For this review, take the finished solid that the model builds, in its own axes (mm). A direction names the side the tool comes from. Round coordinates to 2 decimals unless told otherwise and drop trailing zeros.
from build123d import *

# Parameters (mm, degrees)
FILLET1_R = 40
FILLET2_R = 38
FILLET3_R = 16
FILLET4_R = 4


with BuildPart() as part:
    # Sketch1 → Revolve1 (revolve)
    with BuildSketch(Plane.XY, mode=Mode.PRIVATE) as revolve1_sk:
        Polygon((-150, 1.447982474), (-150, 24.174941718), (-52.599310337, 68.447982474), (0, 68.447982474), (0, 56.447982474), (-50, 56.447982474), (-132, 19.175255201), (-132, 1.447982474), (-132, -4.552017526), (-138, -4.552017526), (-138, 1.447982474), align=None)
    revolve(revolve1_sk.sketch.rotate(Axis((0, 0, 0), (0, 1, 0)), 270), axis=Axis((0, 0, 0), (0, 1, 0)))

    # Fillet1
    fillet1_edges = [part.edges().sort_by_distance(p)[0] for p in [
        (0, 68.447982474, 52.599310337),
    ]]
    fillet(fillet1_edges, radius=FILLET1_R)

    # Fillet2
    fillet2_edges = [part.edges().sort_by_distance(p)[0] for p in [
        (0, 56.447982474, 50),
    ]]
    fillet(fillet2_edges, radius=FILLET2_R)

    # Fillet3
    fillet3_edges = [part.edges().sort_by_distance(p)[0] for p in [
        (0, 24.174941718, 150),
    ]]
    fillet(fillet3_edges, radius=FILLET3_R)

    # Fillet4
    fillet4_edges = [part.edges().sort_by_distance(p)[0] for p in [
        (0, 19.175255201, 132),
    ]]
    fillet(fillet4_edges, radius=FILLET4_R)


solid = part.part
(1) Draft analysis for pull direction Z (two halves, no side actions). For faces 3 (the face through (62.847, 63.094, 13.956)), 4 (the face through (55.01, 50.99, -28.61)), 5 (the face through (122, 1.448, 66)), 6 (the face through (128.86, 6.17, 28.62)), state which applies: pulls with the +Z half, pulls with the -Z half, needs draft (parallel to the pull), parting line crosses it, or undercut.
(2) Tool access review of faces 1 (the face through (91.273, 7.747, 119.035)), 2 (the face through (-6.068, -1.51, 137.867)): name each direction out of +Z, -Z, +X, -X, +Y, -Y from which nothing blocks a thin tool from reaching the whole face with its end or side.
(3) Clearance check with flat-ended pins moving along their axes: P1, Ø4, axis at x = 93.5, z = 39, coming from the -Y side; P2, Ø1.5, axis at y = 24.5, z = -3.5, coming from the -X side; P3, Ø4, axis at x = 26, y = 29, coming from the -Z side; P4, Ø12, axis at x = 113.5, z = -109.5, coming from the -Y side. State where each tip first meets the part, or that it passes through.
(4) Wall thickness on L1, parallel to X at y = 2, z = 0; L2, parallel to X at y = 1, z = 0; L3, parallel to Z at x = -83.5, y = 19.5: over which ranges is each line inside the solid? List them lowest first.
Here are the results:
1. face 3: parting line crosses it
1. face 4: undercut
1. face 5: needs draft
1. face 6: undercut
2. face 1: +Y, -Y
2. face 2: -Y
3. P1: stops at y = 32.22
3. P2: stops at x = -146.55
3. P3: stops at z = -140.79
3. P4: passes through
4. L1: x = -150 to -132, 132 to 150
4. L2: x = -138 to -132, 132 to 138
4. L3: z = -123.38 to -100.62, 100.62 to 123.38
